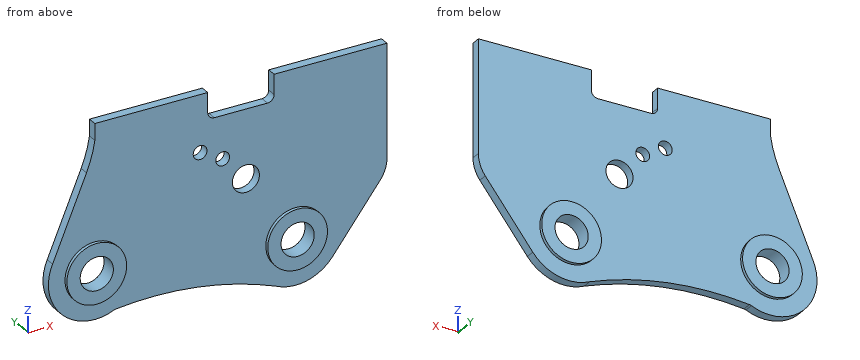
from build123d import *

# Parameters (mm, degrees)
SKETCH1_R             = 20.75
SKETCH1_R_2           = 90
SKETCH1_R_3           = 40.75
BOSS_EXTRUDE1_DEPTH   = 28
SKETCH_2_2_R          = 90
SKETCH_2_2_R_2        = 50
BOSS_EXTRUDE2_DEPTH   = 10
BOSS_EXTRUDE2_2_DEPTH = 10
BOSS_EXTRUDE3_START   = -38
SKETCH_2_2_2_R        = 90
SKETCH_2_2_2_R_2      = 50
BOSS_EXTRUDE3_DEPTH   = 38


with BuildPart() as part:
    # Sketch1 → Boss-Extrude1 (new body)
    with BuildSketch(Plane(origin=(0, 0, 0), x_dir=(1, 0, 0), z_dir=(0, 1, 0))):
        with BuildLine():
            Line((1925.70113656, 1748.394060435), (2027.880227878, 1505.832022369))
            ThreePointArc((2027.880227878, 1505.832022369), (2043.18353175, 1462.087406566), (2052.944070187, 1416.782722365))
            Line((2052.944070187, 1416.782722365), (2052.944070187, 1366.782722365))
            Line((2052.944070187, 1366.782722365), (2392.944070187, 1366.782722365))
            Line((2392.944070187, 1366.782722365), (2392.944070187, 1426.782722365))
            ThreePointArc((2392.944070187, 1426.782722365), (2398.801934564, 1440.924857989), (2412.944070187, 1446.782722365))
            Line((2412.944070187, 1446.782722365), (2572.944070187, 1446.782722365))
            ThreePointArc((2572.944070187, 1446.782722365), (2587.086205811, 1440.924857989), (2592.944070187, 1426.782722365))
            Line((2592.944070187, 1426.782722365), (2592.944070187, 1366.782722365))
            Line((2592.944070187, 1366.782722365), (2932.944070187, 1366.782722365))
            Line((2932.944070187, 1366.782722365), (2932.944070187, 1705.998908982))
            ThreePointArc((2932.944070187, 1705.998908982), (2927.653962259, 1738.093088264), (2912.343343312, 1766.791634101))
            Line((2912.343343312, 1766.791634101), (2769.10349201, 1953.872243723))
            ThreePointArc((2769.10349201, 1953.872243723), (2690.844558049, 2004.841768703), (2597.944509636, 1995.253534964))
            ThreePointArc((2597.944509636, 1995.253534964), (2361.126178322, 1934.317555647), (2116.599187921, 1932.684586999))
            ThreePointArc((2116.599187921, 1932.684586999), (2113.568985738, 1933.277336612), (2110.666130639, 1934.329434346))
            ThreePointArc((2110.666130639, 1934.329434346), (1953.690461842, 1905.518335141), (1925.70113656, 1748.394060435))
        make_face()
        with Locations(Location((2369.944070187, 1538.282722365, 0), (0, 0, 270))):
            Circle(SKETCH1_R, mode=Mode.SUBTRACT)
        with Locations(Location((2437.944070187, 1575.282722365, 0), (0, 0, 270))):
            Circle(SKETCH1_R, mode=Mode.SUBTRACT)
        with Locations(Location((2052.944070187, 1806.782722365, 0), (0, 0, 270))):
            Circle(SKETCH1_R_2, mode=Mode.SUBTRACT)
        with Locations(Location((2657.944509636, 1868.762428557, 0), (0, 0, 270))):
            Circle(SKETCH1_R_2, mode=Mode.SUBTRACT)
        with Locations(Location((2507.944070187, 1652.782722365, 0), (0, 0, 270))):
            Circle(SKETCH1_R_3, mode=Mode.SUBTRACT)
    extrude(amount=BOSS_EXTRUDE1_DEPTH)



with BuildPart() as body_2:
    # Sketch 2_2 → Boss-Extrude2 (new body)
    with BuildSketch(Plane(origin=(0, 28, 0), x_dir=(1, 0, 0), z_dir=(0, 1, 0))):
        with Locations(Location((2052.944070187, 1806.782722365, 0), (0, 0, 270))):
            Circle(SKETCH_2_2_R)
        with Locations(Location((2052.944070187, 1806.782722365, 0), (0, 0, 270))):
            Circle(SKETCH_2_2_R_2, mode=Mode.SUBTRACT)
    extrude(amount=BOSS_EXTRUDE2_DEPTH)


with BuildPart() as body_3:
    # Sketch 2_2 → Boss-Extrude2 2 (new body)
    with BuildSketch(Plane(origin=(0, 28, 0), x_dir=(1, 0, 0), z_dir=(0, 1, 0))):
        with Locations(Location((2657.944509636, 1868.762428557, 0), (0, 0, 270))):
            Circle(SKETCH_2_2_R)
        with Locations(Location((2657.944509636, 1868.762428557, 0), (0, 0, 270))):
            Circle(SKETCH_2_2_R_2, mode=Mode.SUBTRACT)
    extrude(amount=BOSS_EXTRUDE2_2_DEPTH)


with BuildPart() as part_1:
    add(part.part)

    add(body_2.part)  # Boss-Extrude3 merges body 2

    add(body_3.part)  # Boss-Extrude3 merges body 3
    # Sketch 2_2 2 → Boss-Extrude3 (add)
    # profile 1 of 2: a face of its own
    with BuildSketch(Plane(origin=(0, 28, 0), x_dir=(1, 0, 0), z_dir=(0, 1, 0)).offset(BOSS_EXTRUDE3_START)):
        with Locations(Location((2052.944070187, 1806.782722365, 0), (0, 0, 270))):
            Circle(SKETCH_2_2_2_R)
        with Locations(Location((2052.944070187, 1806.782722365, 0), (0, 0, 270))):
            Circle(SKETCH_2_2_2_R_2, mode=Mode.SUBTRACT)
    # profile 2 of 2: a face of its own
    with BuildSketch(Plane(origin=(0, 28, 0), x_dir=(1, 0, 0), z_dir=(0, 1, 0)).offset(BOSS_EXTRUDE3_START)):
        with Locations(Location((2657.944509636, 1868.762428557, 0), (0, 0, 270))):
            Circle(SKETCH_2_2_2_R)
        with Locations(Location((2657.944509636, 1868.762428557, 0), (0, 0, 270))):
            Circle(SKETCH_2_2_2_R_2, mode=Mode.SUBTRACT)
    extrude(amount=BOSS_EXTRUDE3_DEPTH)


solid = part_1.part
Geometry check sheet. Reference: the model listing, model coordinates, mm. Give positions to 0.01 mm unless a question says otherwise; leave off trailing zeros. Order: outer loops, then holes, each group sorted by start corner. A loop starts at its lowest first (then second) coordinate and runs counter-clockwise, first axis right, second up.
1) Cross-section at D-D (z = -1571). Record the boundary of the cut face in (x, y).
Results are:
outline: (2000.43, 0) - (2417.64, 0) - (2417.64, 28) - (2000.43, 28) - close; (2458.25, 0) - (2932.94, 0) - (2932.94, 28) - (2458.25, 28) - close
2) Cross-section at A-A (x = 2690.5). Record the boundary of the cut face in (y, z), then the cut area to 3 significant figures.
Results are:
outline: (-10, -1952.67) - (0, -1952.67) - (0, -2004.92) - (28, -2004.92) - (28, -1952.67) - (38, -1952.67) - (38, -1906.71) - (-10, -1906.71) - close; (-10, -1830.81) - (38, -1830.81) - (38, -1784.86) - (28, -1784.86) - (28, -1366.78) - (0, -1366.78) - (0, -1784.86) - (-10, -1784.86) - close
area: 17,600 mm2
3) Material ranges on probe 1 along Y at (x, z) = (2769, -1589); probe 2 along X at (y, z) = (25, -1836.5); probe 3 along Z at (x, y) = (2014, 23.5), recorded low to high.
Results are:
probe 1: y = 0 to 28
probe 2: x = 1916.13 to 2012.73, 2093.15 to 2619.75, 2696.14 to 2858.97
probe 3: z = -1941.26 to -1838.14, -1775.42 to -1538.78
4) Cross-section at C-C (y = 8). Record the boundary of the cut face in (x, z).
Results are:
outline: (1925.7, -1748.39) arc R140 ccw to (2110.67, -1934.33) arc R20 cw to (2116.6, -1932.68) arc R999.9 cw to (2597.94, -1995.25) arc R140 ccw to (2769.1, -1953.87) - (2912.34, -1766.79) arc R100 ccw to (2932.94, -1706) - (2932.94, -1366.78) - (2592.94, -1366.78) - (2592.94, -1426.78) arc R20 cw to (2572.94, -1446.78) - (2412.94, -1446.78) arc R20 cw to (2392.94, -1426.78) - (2392.94, -1366.78) - (2052.94, -1366.78) - (2052.94, -1416.78) arc R373 cw to (2027.88, -1505.83) - close; hole circle Ø100 at (2052.94, -1806.78); hole circle Ø41.5 at (2369.94, -1538.28); hole circle Ø41.5 at (2437.94, -1575.28); hole circle Ø81.5 at (2507.94, -1652.78); hole circle Ø100 at (2657.94, -1868.76)
5) Gauge pin test, flat ends, axial feed: pin 1 (8 mm diameter, centred on x = 2391, y = 24, fed in from -Z); pin 2 (10 mm diameter, centred on x = 2709, z = -1478, fed in from -Y); pin 3 (22.5 mm diameter, centred on y = 17, z = -1403, fed in from -X). Record the tip position at first contact, or that the pin passes through.
Results are:
pin 1: stops at z = -1939.31
pin 2: stops at y = 0
pin 3: stops at x = 2052.94
6) Cross-section at B-B (z = -1796). Record the boundary of the cut face in (x, y), then the cut area to 3 significant figures.
Results are:
outline: (1913.36, 0) - (1963.59, 0) - (1963.59, -10) - (2004.12, -10) - (2004.12, 38) - (1963.59, 38) - (1963.59, 28) - (1913.36, 28) - close; (2101.77, -10) - (2142.3, -10) - (2142.3, 0) - (2604.98, 0) - (2604.98, -10) - (2710.91, -10) - (2710.91, 0) - (2889.98, 0) - (2889.98, 28) - (2710.91, 28) - (2710.91, 38) - (2604.98, 38) - (2604.98, 28) - (2142.3, 28) - (2142.3, 38) - (2101.77, 38) - close
area: 28,400 mm2
